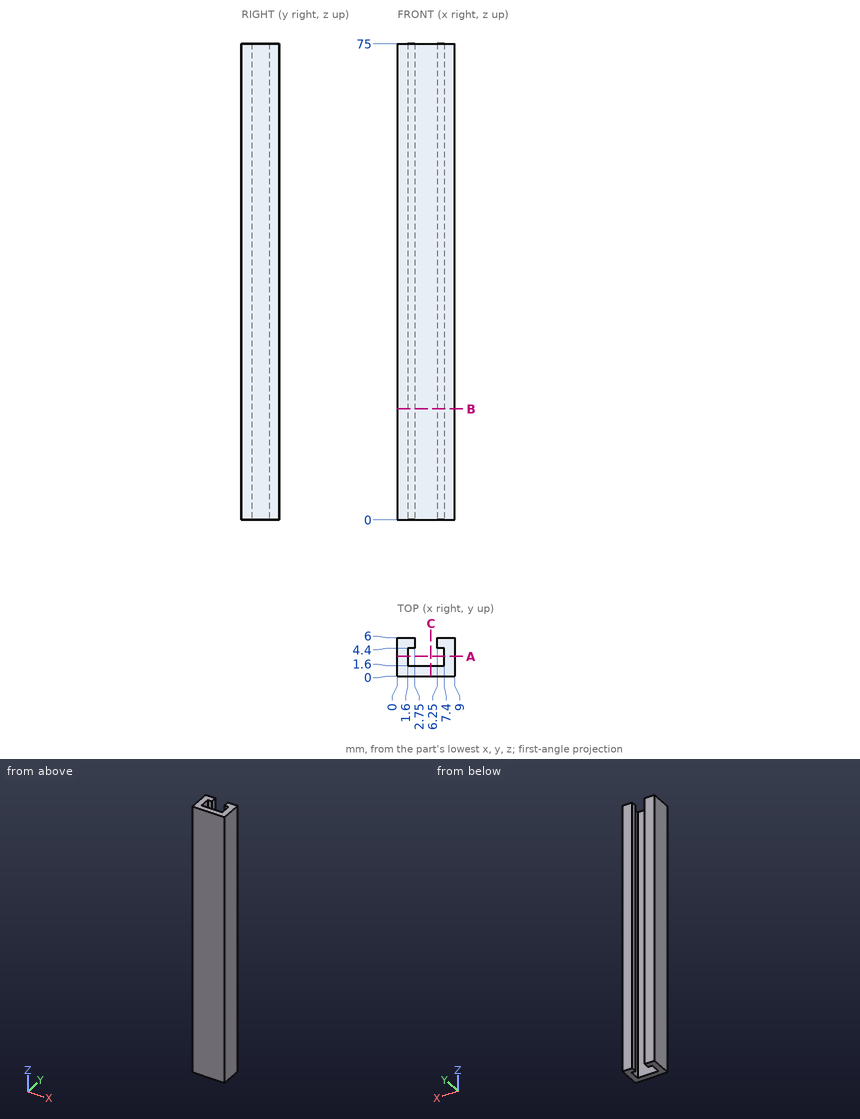
Study the drawing (mm; zero at the part's minimum x, y, z) and answer. Give positions to 0.01 mm unless a question says otherwise; leave off trailing zeros. Write each loop counter-clockwise with the first axis right and the second up, starting at its lowest first coordinate (ties: lowest second). Pieces come first, ordered by that corner, then holes. Notation, with made-up numbers: (72, 27) -> (95, 27) arc R9 cw to (95, 32) -> close; hole circle Ø11 at (23.25, 48.25). An arc over 180 degrees is marked (long way). Answer as a JSON object with one key per item and string values. Group by question number.
1) Find section B-B (z = 17.5). Write down the section's boundary in (x, y).
2) Consider L1, parallel to X at y = 3.8, z = 61.5; L2, parallel to X at y = 5.65, z = 13.5; L3, parallel to Y at x = 3, z = 26. Determine where each line is inside the solid, lowest interval first. Write a range as from..to.
3) Find section C-C (x = 5.25). Write down the section's boundary in (y, z).
4) Each of these flat-tipped pins is pushed along its axis until it touches: P1, Ø1.5, axis at y = 4, z = 49, coming from the -X side; P2, Ø1.7, axis at x = 4, z = 37, coming from the +Y side. Where does it stop, or does it pass through?
5) Find section A-A (y = 3.1). Write down the section's boundary in (x, z).
Values follow:
{
 "1": {"outline": "(0, 0) -> (9, 0) -> (9, 6) -> (6.25, 6) -> (6.25, 4.4) -> (7.4, 4.4) -> (7.4, 1.6) -> (1.6, 1.6) -> (1.6, 4.4) -> (2.75, 4.4) -> (2.75, 6) -> (0, 6) -> close"},
 "2": {"L1": "x = 0..1.6, 7.4..9", "L2": "x = 0..2.75, 6.25..9", "L3": "y = 0..1.6"},
 "3": {"outline": "(0, 0) -> (1.6, 0) -> (1.6, 75) -> (0, 75) -> close"},
 "4": {"P1": "stops at x = 0", "P2": "stops at y = 1.6"},
 "5": {"outline": "(0, 0) -> (1.6, 0) -> (1.6, 75) -> (0, 75) -> close; (7.4, 0) -> (9, 0) -> (9, 75) -> (7.4, 75) -> close"}
}
